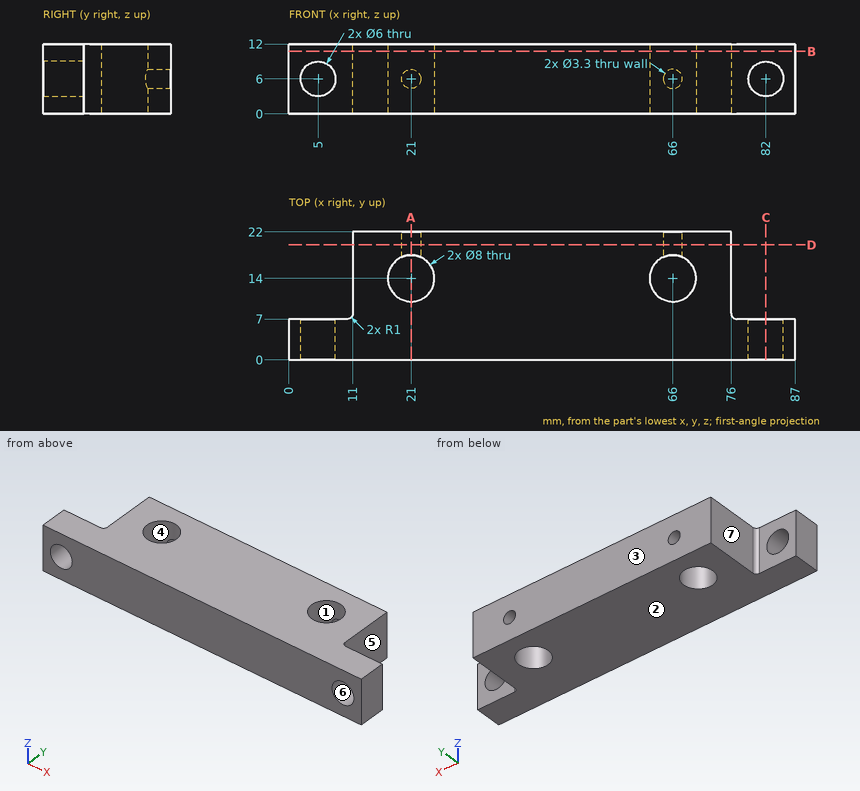
For this review, use the dimensioned drawing (mm, ordinates from the lowest corner) and the shaded views. A direction names the side the tool comes from. Give positions to 0.01 mm unless a question says otherwise; leave off trailing zeros. Loops run counter-clockwise (first coordinate to the right, second up) from the corner with the lowest first, then second, coordinate; pieces in that order, holes last.
Item 1: Take a section at A-A, the plane x = 21. State the section outline as (y, z) points, and give its area (3 significant figures).
Item 2: Take a section at B-B, the plane z = 10.75. State the section outline as (x, y) points, and give its area (3 significant figures).
Item 3: Tool access review of the marked faces 5, 6 and 7: name each direction out of +Z, -Z, +X, -X, +Y, -Y from which nothing blocks a thin tool from reaching the whole face with its end or side.
Item 4: For line 1 along X through (y, z) = (2, 6); line 2 along X through (y, z) = (17, 3); line 3 along Y through (x, z) = (66, 3.25), list the stretches that pass through material, from the lowest coordinate up.
Item 5: Draft analysis for pull direction Y (two halves, no side actions). For the marked faces 1, 2, 3 and 4, state which applies: +Y half, -Y half, draft (parallel to the pull), parting line (faces both ways), or undercut.
Item 6: Insertion check: pin 1 (5 mm diameter, centred on x = 5, z = 6, fed in from +Y); pin 2 (1.5 mm diameter, centred on y = 13.5, z = 10.5, fed in from +X); pin 3 (3 mm diameter, centred on x = 6.5, z = 5, fed in from +Y); pin 4 (3.5 mm diameter, centred on y = 16, z = 9, fed in from -X). Each pin has a flat end and moves straight along its axis. Give the tip position at first contact, or say it passes through.
Item 7: Take a section at D-D, the plane y = 19.75. State the section outline as (x, z) points.
Item 8: Take a section at C-C, the plane x = 82. State the section outline as (y, z) points, and give its area (3 significant figures).
Calculated:
1. outline: (0, 0) - (10, 0) - (10, 12) - (0, 12) - close; (18, 0) - (22, 0) - (22, 4.35) - (18, 4.35) - close; (18, 7.65) - (22, 7.65) - (22, 12) - (18, 12) - close
1. area: 155 mm2
2. outline: (0, 0) - (87, 0) - (87, 7) - (77, 7) arc R1 cw to (76, 8) - (76, 22) - (11, 22) - (11, 8) arc R1 cw to (10, 7) - (0, 7) - close; hole circle Ø8 at (21, 14); hole circle Ø8 at (66, 14)
2. area: 1,480 mm2
3. face 5: +Z, -Z, +X, +Y
3. face 6: +Y, -Y
3. face 7: +Z, -Z, -X, +Y
4. line 1: x = 0 to 2, 8 to 79, 85 to 87
4. line 2: x = 11 to 18.35, 23.65 to 63.35, 68.65 to 76
4. line 3: y = 0 to 10, 18 to 22
5. face 1: undercut
5. face 2: draft
5. face 3: +Y half
5. face 4: undercut
6. pin 1: passes through
6. pin 2: stops at x = 76
6. pin 3: stops at y = 7
6. pin 4: stops at x = 11
7. outline: (11, 0) - (76, 0) - (76, 12) - (11, 12) - close; hole circle Ø3.3 at (21, 6); hole circle Ø3.3 at (66, 6)
8. outline: (0, 0) - (7, 0) - (7, 3) - (0, 3) - close; (0, 9) - (7, 9) - (7, 12) - (0, 12) - close
8. area: 42.0 mm2
